Source: three-view drawing plus pictorial views. Frame: mm from the lowest corner of the part. Round coordinates to 2 decimals unless told otherwise and drop trailing zeros. Write each loop counter-clockwise with the first axis right and the second up, starting at its lowest first coordinate (ties: lowest second). Pieces come first, ordered by that corner, then holes. Notation, with made-up numbers: M 25,-28.5 L 56,-28.5 A9 cw 56,-22.5 Z; hole C 52,-31 d8. An arc over 180 degrees is marked long. Answer in a Markdown table with one row per item.
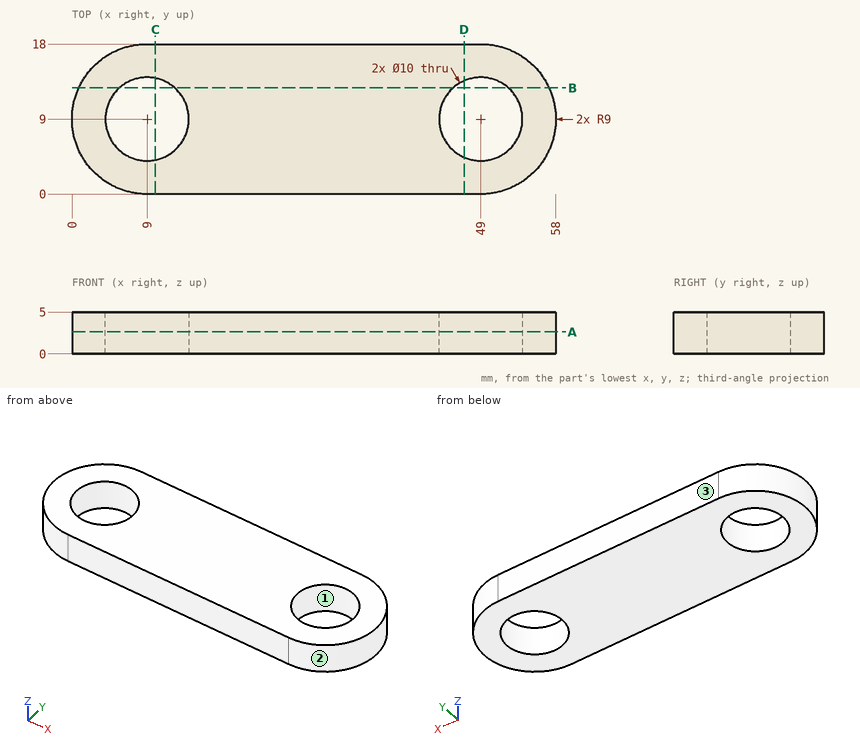
Q1. Section A-A (z = 2.65). Return loops of the section in (x, y).
Solutions:
| item | result |
|---|---|
| outline | M 9,0 L 49,0 A9 ccw 49,18 L 9,18 A9 ccw Z; hole C 9,9 d10; hole C 49,9 d10 |
Q2. Pull-direction query (Y, two-part tool) for the marked faces 1, 2 and 3; classes: pulls with the +Y half, pulls with the -Y half, needs draft (parallel to the pull), parting line crosses it, or undercut.
Solutions:
| item | result |
|---|---|
| face 1 | undercut |
| face 2 | parting line crosses it |
| face 3 | pulls with the +Y half |
Q3. Section C-C (x = 10). Return loops of the section in (y, z), and give its area (3 significant figures).
Solutions:
| item | result |
|---|---|
| outline | M 0,0 L 4.1,0 L 4.1,5 L 0,5 Z; M 13.9,0 L 18,0 L 18,5 L 13.9,5 Z |
| area | 41.0 mm2 |
Q4. Section B-B (y = 12.75). Return loops of the section in (x, z), and give its area (3 significant figures).
Solutions:
| item | result |
|---|---|
| outline | M 0.82,0 L 5.69,0 L 5.69,5 L 0.82,5 Z; M 12.31,0 L 45.69,0 L 45.69,5 L 12.31,5 Z; M 52.31,0 L 57.18,0 L 57.18,5 L 52.31,5 Z |
| area | 216 mm2 |
Q5. Material intervals for probe 1 along X at (y, z) = (5.75, 1.6); probe 2 along Y at (x, z) = (49, 2.75); probe 3 along X at (y, z) = (6, 3.95), sorted ascending.
Solutions:
| item | result |
|---|---|
| probe 1 | x = 0.61 to 5.2, 12.8 to 45.2, 52.8 to 57.39 |
| probe 2 | y = 0 to 4, 14 to 18 |
| probe 3 | x = 0.51 to 5, 13 to 45, 53 to 57.49 |
Q6. Section D-D (x = 47). Return loops of the section in (y, z), and give its area (3 significant figures).
Solutions:
| item | result |
|---|---|
| outline | M 0,0 L 4.42,0 L 4.42,5 L 0,5 Z; M 13.58,0 L 18,0 L 18,5 L 13.58,5 Z |
| area | 44.2 mm2 |
